Could you check a few things on this model? Use its own coordinates, in mm. Face numbers are marked on the shaded views. A direction names the side the tool comes from. Round coordinates to 2 decimals unless told otherwise and drop trailing zeros. Order: outer loops, then holes, each group sorted by start corner. A loop starts at its lowest first (then second) coordinate and runs counter-clockwise, first axis right, second up. Notation, with made-up numbers: (68.5, 16.25) - (120.5, 16.25) arc R14 cw to (120.5, 27.25) - close; hole circle Ø1 at (45.25, 76). An arc over 180 degrees is marked (long way). Use one line per item in the form item = value.
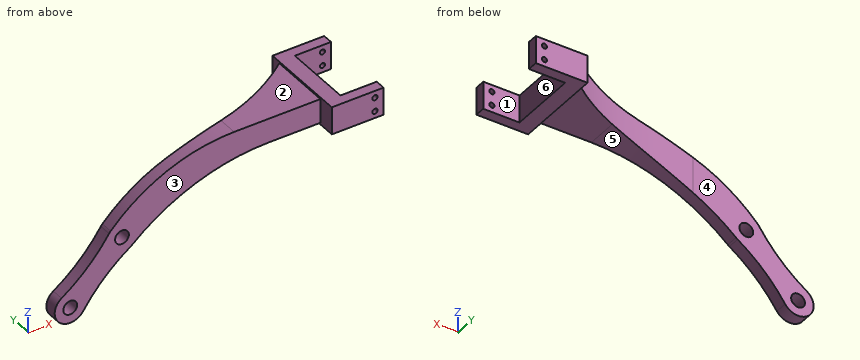
from build123d import *

# Parameters (mm, degrees)
SKETCH1_W           = 150
SKETCH1_H           = 260
BOSS_EXTRUDE1_DEPTH = 40
SKETCH2_W           = 210
SKETCH2_H           = 200
CUT_EXTRUDE1_DEPTH  = 171.073513517
SKETCH3_R           = 20
BOSS_EXTRUDE2_DEPTH = 100
SKETCH4_W           = 803.619965953
SKETCH4_H           = 20
CUT_EXTRUDE2_DEPTH  = 938.629990988
SKETCH5_R           = 7.5
CUT_EXTRUDE3_DEPTH  = 950.025816298


with BuildPart() as part:
    # Sketch1 → Boss-Extrude1 (new, symmetric)
    with BuildSketch(Plane.XY):
        Rectangle(SKETCH1_W, SKETCH1_H)
    extrude(amount=BOSS_EXTRUDE1_DEPTH, both=True)

    # Sketch2 → Cut-Extrude1 (cut, through all)
    with BuildSketch(Plane.XY.offset(40)):
        with Locations((75, 0)):
            Rectangle(SKETCH2_W, SKETCH2_H)
    extrude(amount=-CUT_EXTRUDE1_DEPTH, mode=Mode.SUBTRACT)

    # Sketch3 → Boss-Extrude2 (add, symmetric)
    with BuildSketch(Plane(origin=(0, 0, 0), x_dir=(1, 0, 0), z_dir=(0, 1, 0))):
        with BuildLine():
            Line((-75, 35), (-75, -35))
            Line((-75, -35), (-325, -35))
            ThreePointArc((-325, -35), (-519.738798114, 5.159932949), (-682.701137952, 119.086644041))
            ThreePointArc((-682.701137952, 119.086644041), (-685.176285552, 121.935272409), (-687.404051985, 124.981269115))
            ThreePointArc((-687.404051985, 124.981269115), (-749.451239008, 200.548760992), (-825.018730885, 262.595948015))
            ThreePointArc((-825.018730885, 262.595948015), (-831.819805153, 331.819805153), (-762.595948015, 325.018730885))
            ThreePointArc((-762.595948015, 325.018730885), (-700.548760992, 249.451239008), (-624.981269115, 187.404051985))
            ThreePointArc((-624.981269115, 187.404051985), (-622.594074072, 185.691949008), (-620.323675597, 183.827736695))
            ThreePointArc((-620.323675597, 183.827736695), (-436.205174947, 73.439379047), (-225, 35))
            Line((-225, 35), (-75, 35))
        make_face()
        with Locations(Location((-800, 300, 0), (0, 0, 270))):
            Circle(SKETCH3_R, mode=Mode.SUBTRACT)
        with Locations(Location((-650, 150, 0), (0, 0, 270))):
            Circle(SKETCH3_R, mode=Mode.SUBTRACT)
    extrude(amount=BOSS_EXTRUDE2_DEPTH, both=True)

    # Sketch4 → Cut-Extrude2 (cut, through all)
    with BuildSketch(Plane.XY.offset(40)):
        with BuildLine():
            Line((-845, -43.779068644), (-495, -43.779068644))
            ThreePointArc((-495, -43.779068644), (-273.03580211, -6.838732152), (-75, 100))
            Line((-75, 100), (-75, 271.543377567))
            Line((-75, 271.543377567), (-940.801447503, 271.543377567))
            Line((-940.801447503, 271.543377567), (-972.091183845, -20.942543752))
            Line((-972.091183845, -20.942543752), (-845, -43.779068644))
        make_face()
        with Locations((-476.809982977, -90)):
            Rectangle(SKETCH4_W, SKETCH4_H)
    extrude(amount=-CUT_EXTRUDE2_DEPTH, mode=Mode.SUBTRACT)

    # Sketch5 → Cut-Extrude3 (cut, through all)
    with BuildSketch(Plane(origin=(0, 130, 0), x_dir=(1, 0, 0), z_dir=(0, 1, 0))):
        with Locations(Location((50, 20, 0), (0, 0, 270))):
            Circle(SKETCH5_R)
        with Locations(Location((50, -20, 0), (0, 0, 270))):
            Circle(SKETCH5_R)
    extrude(amount=-CUT_EXTRUDE3_DEPTH, mode=Mode.SUBTRACT)


solid = part.part
Item 1: I need wall thicknesses on L1, parallel to X at y = -121.25, z = 20; L2, parallel to Y at x = -704, z = -227; L3, parallel to Z at x = -46.5, y = -4. Which ranges of each line are inside material? Lowest first, please.
Found:
L1 = -75 to 42.5, 57.5 to 75
L2 = -80 to -43.78
L3 = -40 to 40
Item 2: For the marked faces 4, 5 and 6, which set-ups out of +Z, -Z, +X, -X, +Y, -Y let a thin tool reach every point of the face, with its end or its side?
Found:
face_4 = +Z, -Z, -X, +Y
face_5 = -Z, +Y, -Y
face_6 = +Z, -Z, +X
Item 3: If we mould it in two halves opening along Y, with no side actions, what happens to the marked faces 1, 2 and 3? For each: released by +Y, released by -Y, zero draft, split by the parting line, or undercut.
Found:
face_1 = undercut
face_2 = zero draft
face_3 = released by -Y
Item 4: Imagine slicing it at C-C on y = 78.5. Please give me the cut outline in (x, z).
Found:
outline = (-104.29, -35) - (-75, -35) - (-75, -40) - (-30, -40) - (-30, 40) - (-75, 40) - (-75, 35) - (-104.29, 35) - close
Item 5: Imagine slicing it at B-B on z = -300. Please give me the cut outline in (x, y), plus the area to 3 significant figures.
Found:
outline = (-845, -80) - (-820, -80) - (-820, -43.78) - (-845, -43.78) - close; (-780, -80) - (-744.72, -80) - (-744.72, -43.78) - (-780, -43.78) - close
area = 2,180 mm2
Item 6: Imagine slicing it at D-D on x = -410. Please give me the cut outline in (y, z).
Found:
outline = (-80, -64.26) - (-38.49, -64.26) - (-38.49, 27.61) - (-80, 27.61) - close
Item 7: Will these pins go through, and if not, where does the flat tip stop? P1, Ø1.5, axis at x = -110.5, y = -45, coming from the +Z side; P2, Ø2, axis at y = -0.5, z = -6.5, coming from the +X side.
Found:
P1 = 35
P2 = -30
Item 8: Imagine slicing it at A-A on x = 10.5. Please give me the cut outline in (y, z).
Found:
outline = (-130, -40) - (-100, -40) - (-100, 40) - (-130, 40) - close; (100, -40) - (130, -40) - (130, 40) - (100, 40) - close
